from build123d import *

# Parameters (mm, degrees)
BASE_PLATE_SKETCH_W             = 160
BASE_PLATE_SKETCH_H             = 100
BASE_PLATE_160X100X15_DEPTH     = 15
BASE_PLATE_CORNER_FILLETS_R15_R = 15
MOUNTING_HOLES_SKETCH_R         = 6
MOUNTING_HOLES_4X_12_DEPTH      = 15
INCLINED_ARM_PROFILE_SKETCH_R   = 15
INCLINED_ARM_PROFILE_SKETCH_R_2 = 6.5
INCLINED_ARM_DEPTH              = 15
ARM_SUPPORT_WEB_REACH           = 134.937
ARM_SUPPORT_WEB_SKETCH_R        = 15


with BuildPart() as part:
    # Base Plate Sketch → Base Plate 160x100x15 (new body)
    with BuildSketch(Plane(origin=(0, 0, 0), x_dir=(1, 0, 0), z_dir=(0, 1, 0))):
        Rectangle(BASE_PLATE_SKETCH_W, BASE_PLATE_SKETCH_H)
    extrude(amount=BASE_PLATE_160X100X15_DEPTH)

    # Base Plate Corner Fillets R15
    base_plate_corner_fillets_r15_edges = [part.edges().sort_by_distance(p)[0] for p in [
        (80, 7.5, 50),
        (-80, 7.5, 50),
        (-80, 7.5, -50),
        (80, 7.5, -50),
    ]]
    fillet(base_plate_corner_fillets_r15_edges, radius=BASE_PLATE_CORNER_FILLETS_R15_R)

    # Mounting Holes Sketch → Mounting Holes 4x_12 (cut)
    with BuildSketch(Plane(origin=(0, 15, 0), x_dir=(1, 0, 0), z_dir=(0, 1, 0))):
        with Locations(Location((-65, 35, 0), (0, 0, 270))):
            Circle(MOUNTING_HOLES_SKETCH_R)
        with Locations(Location((65, 35, 0), (0, 0, 270))):
            Circle(MOUNTING_HOLES_SKETCH_R)
        with Locations(Location((65, -35, 0), (0, 0, 270))):
            Circle(MOUNTING_HOLES_SKETCH_R)
        with Locations(Location((-65, -35, 0), (0, 0, 270))):
            Circle(MOUNTING_HOLES_SKETCH_R)
    extrude(amount=-MOUNTING_HOLES_4X_12_DEPTH, mode=Mode.SUBTRACT)

    # Arm Support Web: up to this face of the body (flat: up to its plane)
    arm_support_web_end = Plane(part.part.faces().sort_by_distance((0, 15, 0))[0])
    # Arm Support Web Sketch → Arm Support Web (add, up to the picked face)
    with BuildSketch(Plane(origin=(26.495190528, 45.891016151, 0), x_dir=(0.8660254037844417, -0.4999999999999947, 0), z_dir=(0.4999999999999947, 0.8660254037844417, 0)), mode=Mode.PRIVATE) as arm_support_web_sk1:
        with BuildLine():
            Line((61.782032303, 7.5), (61.782032303, -7.5))
            Line((61.782032303, -7.5), (-11.591402841, -7.5))
            ThreePointArc((-11.591402841, -7.5), (-60.439882876, 0), (-11.591402841, 7.5))
            Line((-11.591402841, 7.5), (61.782032303, 7.5))
        make_face()
        with Locations(Location((-35.439882876, 0, 0), (0, 0, 180))):
            Circle(ARM_SUPPORT_WEB_SKETCH_R, mode=Mode.SUBTRACT)
    arm_support_web_tool1 = split(extrude(arm_support_web_sk1.sketch, amount=-ARM_SUPPORT_WEB_REACH, mode=Mode.PRIVATE), bisect_by=arm_support_web_end, keep=Keep.BOTH, mode=Mode.PRIVATE)


with BuildPart() as body_2:
    # Inclined Arm Profile Sketch → Inclined Arm (new body)
    with BuildSketch(Plane(origin=(26.495190528, 45.891016151, 0), x_dir=(-0.8660254037844417, 0.4999999999999947, 0), z_dir=(0.4999999999999947, 0.8660254037844417, 0))):
        with BuildLine():
            Line((-61.782032303, -17.5), (-5.79117338, -17.5))
            ThreePointArc((-5.79117338, -17.5), (0.755363327, -19.003968837), (5.989128407, -23.214285714))
            ThreePointArc((5.989128407, -23.214285714), (9.720912357, -27.290741204), (14.011311447, -30.774442749))
            ThreePointArc((14.011311447, -30.774442749), (18.735961782, -36.140569101), (20.439882876, -43.084219849))
            Line((20.439882876, -43.084219849), (20.439882876, -50))
            ThreePointArc((20.439882876, -50), (35.439882876, -65), (50.439882876, -50))
            Line((50.439882876, -50), (50.439882876, -43.084219849))
            ThreePointArc((50.439882876, -43.084219849), (52.14380397, -36.140569101), (56.868454305, -30.774442749))
            ThreePointArc((56.868454305, -30.774442749), (62.73062408, 25.718970519), (5.989128407, 23.214285714))
            ThreePointArc((5.989128407, 23.214285714), (0.755363327, 19.003968837), (-5.79117338, 17.5))
            Line((-5.79117338, 17.5), (-61.782032303, 17.5))
            Line((-61.782032303, 17.5), (-61.782032303, -17.5))
        make_face()
        with Locations((35.439882876, 0)):
            Circle(INCLINED_ARM_PROFILE_SKETCH_R, mode=Mode.SUBTRACT)
        with Locations((35.439882876, -50)):
            Circle(INCLINED_ARM_PROFILE_SKETCH_R_2, mode=Mode.SUBTRACT)
    extrude(amount=-INCLINED_ARM_DEPTH)


with BuildPart() as part_1:
    add(part.part)

    add(body_2.part)  # Arm Support Web merges body 2
    add(arm_support_web_tool1.solids().sort_by(Axis((20.297634, 49.469177, 0), (-0.4999999999999947, -0.8660254037844417, 0)))[0])


solid = part_1.part
Here's how the part is built. I have some questions about the finished solid (model axes, mm). A direction names the side the tool comes from. Give positions to 0.01 mm unless a question says otherwise; leave off trailing zeros. One line per item, written item: value. Start each with the question number.
1. I need wall thicknesses on probe 1 along X at (y, z) = (7, -35); probe 2 along X at (y, z) = (39, 12.5); probe 3 along Y at (x, z) = (-47, 32). Which ranges of each line are inside material? Lowest first, please. Write a range as from..to.
2. Imagine slicing it at A-A, the plane x = -38.5. Count the separate pieces of the cut face and the enclosed holes in it, plus the area to 3 significant figures.
3. Will these pins go through, and if not, where does the flat tip stop? pin 1 Ø8 at (x, z) = (63, -48.5) entering from -Y; pin 2 Ø4.5 at (x, y) = (-29, 10) entering from -Z; pin 3 Ø19 at (x, z) = (65, 35) entering from +Y; pin 4 Ø7 at (x, z) = (-65, -35) entering from -Y.
4. For faces 1 (the face through (-20.885, 64.707, -46.591)), 2 (the face through (5.1, 49.71, -46.49)), 3 (the face through (17, 26, 7.5)), 4 (the face through (6.621, 40.045, -17.307)), which set-ups out of +Z, -Z, +X, -X, +Y, -Y let a thin tool reach every point of the face, with its end or its side?
5. We'd pull the mould along Z, two halves only. Please class faces 5 (the face through (-32.56, 43.1, 4.51)), 6 (the face through (-8, 57, -65)), 7 (the face through (-80, 7, 0)): released by +Z, released by -Z, zero draft, split by the parting line, or undercut.
Values follow:
1. probe 1: x = -80..-71, -59..59, 71..80
1. probe 2: x = -43.41..-27.98, -8.83..6.59, 8.43..38.43
1. probe 3: y = 0..15
2. separate pieces: 2
2. enclosed holes: 1
2. area: 2,910 mm2
3. pin 1: stops at y = 0
3. pin 2: stops at z = -50
3. pin 3: stops at y = 15
3. pin 4: passes through
4. face 1: -Z, -X, +Y
4. face 2: -Z, +X
4. face 3: +Z
4. face 4: none
5. face 5: undercut
5. face 6: released by -Z
5. face 7: zero draft
